Verification items for the finished model (mm, model axes). A direction names the side the tool comes from. Coordinates: 2 decimals unless noted, no trailing zeros. Order: outer loops, then holes, each group sorted by start corner. A loop starts at its lowest first (then second) coordinate and runs counter-clockwise, first axis right, second up. Notation, with made-up numbers: (36.5, 58.5) -> (59.5, 58.5) arc R33 cw to (59.5, 86.5) -> close; hole circle Ø3 at (40.25, -0.75). An arc over 180 degrees is marked (long way). Answer as CSV lines item,"result".
```python
from build123d import *

# Parameters (mm, degrees)
GB_6728_1986_050_X_50_X_3_1_DEPTH = 1050


with BuildPart() as part:
    # Sketch1 → Gb／6728-1986方形空心型钢 050 X 50 X 3(1) (new body)
    with BuildSketch(Plane.YX.offset(-525)):
        with BuildLine():
            Line((-19, -25), (19, -25))
            ThreePointArc((19, -25), (23.242640687, -23.242640687), (25, -19))
            Line((25, -19), (25, 19))
            ThreePointArc((25, 19), (23.242640687, 23.242640687), (19, 25))
            Line((19, 25), (-19, 25))
            ThreePointArc((-19, 25), (-23.242640687, 23.242640687), (-25, 19))
            Line((-25, 19), (-25, -19))
            ThreePointArc((-25, -19), (-23.242640687, -23.242640687), (-19, -25))
        make_face()
        with BuildLine():
            Line((-19, -22), (19, -22))
            ThreePointArc((19, -22), (21.121320344, -21.121320344), (22, -19))
            Line((22, -19), (22, 19))
            ThreePointArc((22, 19), (21.121320344, 21.121320344), (19, 22))
            Line((19, 22), (-19, 22))
            ThreePointArc((-19, 22), (-21.121320344, 21.121320344), (-22, 19))
            Line((-22, 19), (-22, -19))
            ThreePointArc((-22, -19), (-21.121320344, -21.121320344), (-19, -22))
        make_face(mode=Mode.SUBTRACT)
    extrude(amount=GB_6728_1986_050_X_50_X_3_1_DEPTH)


solid = part.part
```
Item 1: Depth check by flat-ended pin: pin 1 Ø12 at (x, y) = (15.5, 9) entering from +Z. Enter the tip coordinate at first touch or a pass-through.
Answer list:
pin 1,"through"
Item 2: Tool access check on faces 4 (the flat face through (0.1, -22.3, 525)), 5 (the flat face through (-22, 0, 7)). Record the directions out of +Z, -Z, +X, -X, +Y, -Y that give a thin tool (end or side, any length) a straight path to the whole face; none if there is none.
Answer list:
face 4,"+Z, +X, -X, +Y, -Y"
face 5,"+Z, -Z"
Item 3: Thickness scan on line 1 (X direction, y = 9, z = -296); line 2 (X direction, y = 20.5, z = 257). Record the ranges inside material, lowest first.
Answer list:
line 1,"-25 to -22, 22 to 25"
line 2,"-24.81 to -21.6, 21.6 to 24.81"
Item 4: Section check A-A, the plane z = 74. Record the boundary of the cut face in (x, y).
Answer list:
outline,"(-25, -19) arc R6 ccw to (-19, -25) -> (19, -25) arc R6 ccw to (25, -19) -> (25, 19) arc R6 ccw to (19, 25) -> (-19, 25) arc R6 ccw to (-25, 19) -> close; hole (-22, -19) arc R3 ccw to (-19, -22) -> (19, -22) arc R3 ccw to (22, -19) -> (22, 19) arc R3 ccw to (19, 22) -> (-19, 22) arc R3 ccw to (-22, 19) -> close"
Item 5: Release check for a two-part mould opening along Y. For faces 1 (the flat face through (22, 0, 7)), 2 (the flat face through (0, -25, 7)), 3 (the flat face through (0, 25, 7)) record: +Y half, -Y half, draft (parallel to the pull), parting line (faces both ways), or undercut.
Answer list:
face 1,"undercut"
face 2,"-Y half"
face 3,"+Y half"
Item 6: Section check B-B, the plane y = 10.5. Record the boundary of the cut face in (x, z).
Answer list:
outline,"(-25, -525) -> (-22, -525) -> (-22, 525) -> (-25, 525) -> close; (22, -525) -> (25, -525) -> (25, 525) -> (22, 525) -> close"
